```python
from build123d import *

# Parameters (mm, degrees)
BASE_PROFILE_10MM_DEPTH = 10
UPPER_BLOCK_30MM_DEPTH  = 30
PAD_SKETCH_W            = 44
PAD_SKETCH_H            = 20
PAD_4MM_DEPTH           = 4
PROFILE_CUT_34MM_DEPTH  = 34
SIDE_WALL_21MM_DEPTH    = 21
RAIL_SKETCH_W           = 40
RAIL_SKETCH_H           = 10
RAIL_5MM_DEPTH          = 5
LUG_BOSS_10MM_DEPTH     = 10
LUG_HOLE_SKETCH_21_R    = 10.5
LUG_HOLE_21_DEPTH       = 10


with BuildPart() as part:
    # Base Profile Sketch → Base Profile 10mm (new body)
    with BuildSketch(Plane.XY):
        with BuildLine():
            Line((40, -55), (22, -55))
            Line((22, -55), (22, -25))
            Line((22, -25), (-22, -25))
            Line((-22, -25), (-22, -55))
            Line((-22, -55), (-40, -55))
            ThreePointArc((-40, -55), (-47.071067812, -52.071067812), (-50, -45))
            Line((-50, -45), (-50, 0))
            Line((-50, 0), (0, 0))
            Line((0, 0), (50, 0))
            Line((50, 0), (50, -45))
            ThreePointArc((50, -45), (47.071067812, -52.071067812), (40, -55))
        make_face()
    extrude(amount=BASE_PROFILE_10MM_DEPTH)

    # Upper Block Sketch → Upper Block 30mm (add)
    with BuildSketch(Plane.XZ.offset(25)):
        Polygon((-22, 10), (-22, 30), (22, 30), (22, 10), (22, 0), (-22, 0), align=None)
    extrude(amount=UPPER_BLOCK_30MM_DEPTH)

    # Pad Sketch → Pad 4mm (add)
    with BuildSketch(Plane(origin=(0, -25, 0), x_dir=(1, 0, 0), z_dir=(0, 1, 0))):
        with Locations((0, -20)):
            Rectangle(PAD_SKETCH_W, PAD_SKETCH_H)
    extrude(amount=PAD_4MM_DEPTH)

    # Profile Cut Sketch → Profile Cut 34mm (cut)
    with BuildSketch(Plane.XZ.offset(55)):
        with BuildLine():
            Line((-20, 0), (20, 0))
            ThreePointArc((20, 0), (0, 20), (-20, 0))
        make_face()
    extrude(amount=-PROFILE_CUT_34MM_DEPTH, mode=Mode.SUBTRACT)

    # Side Wall Sketch → Side Wall 21mm (add)
    with BuildSketch(Plane(origin=(0, 0, 0), x_dir=(1, 0, 0), z_dir=(0, 1, 0))):
        Polygon((0, -55), (20, -55), (50, -10), (-50, -10), (-20, -55), align=None)
    extrude(amount=-SIDE_WALL_21MM_DEPTH)

    # Rail Sketch → Rail 5mm (add)
    with BuildSketch(Plane.XZ.offset(21)):
        with Locations((0, 50)):
            Rectangle(RAIL_SKETCH_W, RAIL_SKETCH_H)
    extrude(amount=RAIL_5MM_DEPTH)

    # Lug Sketch → Lug Boss 10mm (add)
    with BuildSketch(Plane.XY.offset(55)):
        with BuildLine():
            Line((-20, -26), (20, -26))
            ThreePointArc((20, -26), (0, -46), (-20, -26))
        make_face()
    extrude(amount=-LUG_BOSS_10MM_DEPTH)

    # Lug Hole Sketch Ø21 → Lug Hole Ø21 (cut)
    with BuildSketch(Plane.XY.offset(55)):
        with Locations((0, -26)):
            Circle(LUG_HOLE_SKETCH_21_R)
    extrude(amount=-LUG_HOLE_21_DEPTH, mode=Mode.SUBTRACT)


solid = part.part
```
Here's how the part is built. I have some questions about the finished solid (model axes, mm). A direction names the side the tool comes from. Round coordinates to 2 decimals unless told otherwise and drop trailing zeros. Order: outer loops, then holes, each group sorted by start corner. A loop starts at its lowest first (then second) coordinate and runs counter-clockwise, first axis right, second up. Notation, with made-up numbers: M 73.5,19 L 107.5,19 A27 ccw 107.5,56 Z; hole C -27.75,-21 d3. An arc over 180 degrees is marked long. Answer in a Markdown table with one row per item.
Item 1: Thinking about a two-plate mould opening in Y: for faces 6 (the face through (0, -46, 50)), 7 (the face through (22, -38, 20)), 8 (the face through (-1.37, -15.59, 50.07)), which applies, +Y half, -Y half, draft (parallel to the pull), parting line (faces both ways), or undercut?
A:
| item | result |
|---|---|
| face 6 | -Y half |
| face 7 | draft |
| face 8 | undercut |
Item 2: For faces 1 (the face through (0, -19, 45)), 2 (the face through (20, -23, 50)), 3 (the face through (0, -21, 8)), 4 (the face through (-20, -23, 50)), 5 (the face through (0, -38, 30)), which set-ups out of +Z, -Z, +X, -X, +Y, -Y let a thin tool reach every point of the face, with its end or its side?
A:
| item | result |
|---|---|
| face 1 | +Z |
| face 2 | +Z, +X, -Y |
| face 3 | -Z, -Y |
| face 4 | +Z, -X, -Y |
| face 5 | +X, -X, -Y |
Item 3: Imagine slicing it at D-D, the plane z = 5. Write out the boundary of the cut face in (x, y), and give its area (3 significant figures).
A:
| item | result |
|---|---|
| outline | M -50,-45 A10 ccw -40,-55 L -19.36,-55 L -19.36,-21 L 19.36,-21 L 19.36,-55 L 40,-55 A10 ccw 50,-45 L 50,0 L -50,0 Z |
| area | 4,140 mm2 |
Item 4: Imagine slicing it at B-B, the plane x = 0. Write out the boundary of the cut face in (y, z).
A:
| item | result |
|---|---|
| outline | M -55,20 L -21,20 L -21,0 L 0,0 L 0,55 L -15.5,55 L -15.5,45 L -21,45 L -21,30 L -55,30 Z; M -46,45 L -36.5,45 L -36.5,55 L -46,55 Z |
Item 5: Imagine slicing it at A-A, the plane z = 49. Write out the boundary of the cut face in (x, y), and give its area (3 significant figures).
A:
| item | result |
|---|---|
| outline | M -24,-21 L -20,-21 L -20,-26 A20 ccw 20,-26 L 20,-21 L 24,-21 L 24,0 L -24,0 Z; hole C 0,-26 d21 |
| area | 1,490 mm2 |
Item 6: I'm going to push flat-ended pins straight in: pin 1 (12.5 mm diameter, centred on x = 9.5, y = -32, fed in from -Z); pin 2 (22.5 mm diameter, centred on x = 20, z = 35, fed in from -Y); pin 3 (4.5 mm diameter, centred on x = -2.5, y = -19, fed in from +Z); pin 4 (3 mm diameter, centred on y = -12, z = 26, fed in from +X). Where does each tip first touch, or does it pass through?
A:
| item | result |
|---|---|
| pin 1 | stops at z = 12.33 |
| pin 2 | stops at y = -55 |
| pin 3 | stops at z = 45 |
| pin 4 | stops at x = 40.33 |
Item 7: If I drill on L1, parallel to X at y = -26, z = 48; L2, parallel to Y at x = 0, z = 50; L3, parallel to Y at x = 20, z = 34, over which ranges is the centre line in solid material (lowest first)? Write a range as from..to.
A:
| item | result |
|---|---|
| L1 | x = -20..-10.5, 10.5..20 |
| L2 | y = -46..-36.5, -15.5..0 |
| L3 | y = -21..0 |
Item 8: Imagine slicing it at C-C, the plane y = -42.5. Write out the boundary of the cut face in (x, z).
A:
| item | result |
|---|---|
| outline | M -50,0 L -20,0 A20 cw 20,0 L 50,0 L 50,10 L 22,10 L 22,30 L -22,30 L -22,10 L -50,10 Z; M -11.3,45 L 11.3,45 L 11.3,55 L -11.3,55 Z |
